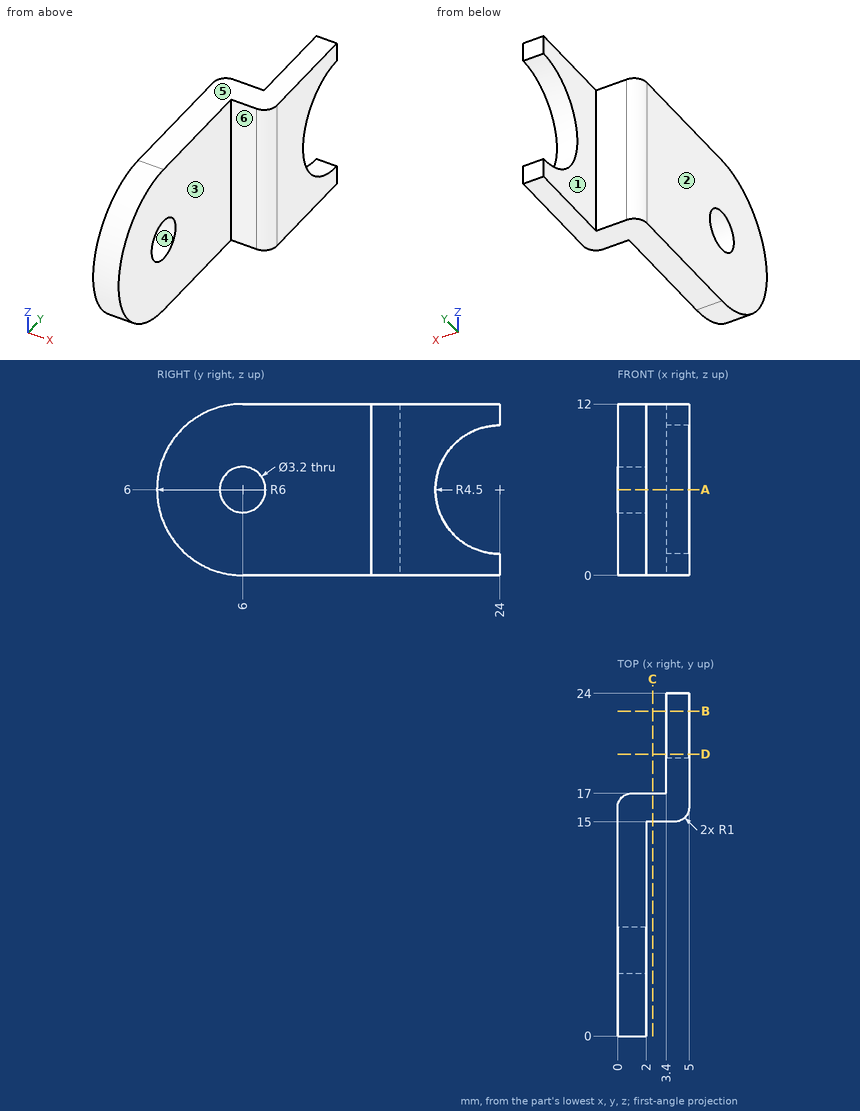
Verification items for this drawing (mm, ordinates from the low corner). A direction names the side the tool comes from. Give positions to 0.01 mm unless a question says otherwise; leave off trailing zeros. Loops run counter-clockwise (first coordinate to the right, second up) from the corner with the lowest first, then second, coordinate; pieces in that order, holes last. Notation, with made-up numbers: M 79,44 L 133,44 A13 cw 133,62 Z; hole C 82.25,-12.5 d5. An arc over 180 degrees is marked long. Write each question's results on one line, items separated by ' | '.
1) Section check B-B, the plane y = 22.75. Record the boundary of the cut face in (x, z).
Answers follow:
outline: M 3.4,0 L 5,0 L 5,1.68 L 3.4,1.68 Z; M 3.4,10.32 L 5,10.32 L 5,12 L 3.4,12 Z
2) Tool access check on the marked faces 1, 2 and 3. Record the directions out of +Z, -Z, +X, -X, +Y, -Y that give a thin tool (end or side, any length) a straight path to the whole face; none if there is none.
Answers follow:
face 1: +Z, -Z, -X, +Y | face 2: +Z, -Z, -X, +Y, -Y | face 3: +Z, -Z, +X, -Y
3) Section check D-D, the plane y = 19.75. Record the boundary of the cut face in (x, z), plus the area to 3 significant figures.
Answers follow:
outline: M 3.4,0 L 5,0 L 5,4.52 L 3.4,4.52 Z; M 3.4,7.48 L 5,7.48 L 5,12 L 3.4,12 Z | area: 14.5 mm2
4) Release check for a two-part mould opening along Z. For the marked faces 4, 5 and 6 record: +Z half, -Z half, draft (parallel to the pull), parting line (faces both ways), or undercut.
Answers follow:
face 4: undercut | face 5: +Z half | face 6: draft
5) Section check C-C, the plane x = 2.45. Record the boundary of the cut face in (y, z), plus the area to 3 significant figures.
Answers follow:
outline: M 15,0 L 17,0 L 17,12 L 15,12 Z | area: 24.0 mm2
6) Gauge pin test, flat ends, axial feed: pin 1 (3 mm diameter, centred on y = 15.5, z = 2, fed in from +X); pin 2 (1 mm diameter, centred on x = 3.5, z = 4.5, fed in from -Y); pin 3 (1.2 mm diameter, centred on x = 1.5, z = 7.5, fed in from +Y). Record the tip position at first contact, or that the pin passes through.
Answers follow:
pin 1: x = 5 | pin 2: y = 15 | pin 3: y = 17
7) Thickness scan on line 1 (Z direction, x = 1, y = 6); line 2 (Y direction, x = 2.9, z = 7.25); line 3 (X direction, y = 11.5, z = 4). Record the ranges inside material, lowest first.
Answers follow:
line 1: 0 to 4.4, 7.6 to 12 | line 2: 15 to 17 | line 3: 0 to 2
8) Section check A-A, the plane z = 6. Record the boundary of the cut face in (x, y), plus the area to 3 significant figures.
Answers follow:
outline: M 0,0 L 2,0 L 2,4.4 L 0,4.4 Z; M 0,7.6 L 2,7.6 L 2,15 L 4,15 A1 ccw 5,16 L 5,19.5 L 3.4,19.5 L 3.4,17 L 1,17 A1 ccw 0,16 Z | area: 37.2 mm2
